```python
from build123d import *

# Parameters (mm, degrees)
SKETCH1_R           = 15
BOSS_EXTRUDE1_DEPTH = 300
SKETCH3_R           = 15
BOSS_EXTRUDE2_DEPTH = 50
BOSS_EXTRUDE3_START = -300
SKETCH5_R           = 15
BOSS_EXTRUDE3_DEPTH = 300


with BuildPart() as part:
    # Sketch1 → Boss-Extrude1 (new, symmetric)
    with BuildSketch(Plane.XY):
        Circle(SKETCH1_R)
    extrude(amount=BOSS_EXTRUDE1_DEPTH, both=True)

    # Sketch2 → Revolve1 (revolve)
    with BuildSketch(Plane(origin=(0, 0, 0), x_dir=(1, 0, 0), z_dir=(0, 1, 0))):
        with BuildLine():
            Line((0, 355), (0, 295))
            ThreePointArc((0, 295), (30, 325), (0, 355))
        make_face()
    revolve1 = revolve(axis=Axis((0, 0, -355), (0, 0, 1)))

    # Mirror1: Revolve1 across plane
    add(revolve1.mirror(Plane.XY))

    # Sketch3 → Boss-Extrude2 (add)
    with BuildSketch(Plane(origin=(0, 0, 0), x_dir=(1, 0, 0), z_dir=(0, 1, 0))):
        Circle(SKETCH3_R)
    extrude(amount=BOSS_EXTRUDE2_DEPTH)

    # Sketch4 → Revolve2 (revolve)
    with BuildSketch(Plane.XY):
        with BuildLine():
            Line((0, 105), (0, 45))
            ThreePointArc((0, 45), (30, 75), (0, 105))
        make_face()
    revolve(axis=Axis((0, 105, 0), (0, -1, 0)))

    # Sketch5 → Boss-Extrude3 (add)
    with BuildSketch(Plane(origin=(0, 0, 0), x_dir=(1, 0, 0), z_dir=(0, 1, 0)).offset(BOSS_EXTRUDE3_START)):
        Circle(SKETCH5_R)
    extrude(amount=BOSS_EXTRUDE3_DEPTH)

    # Sketch6 → Revolve3 (revolve)
    with BuildSketch(Plane(origin=(0, 0, 0), x_dir=(0, 0, -1), z_dir=(1, 0, 0))):
        with BuildLine():
            Line((0, -295), (0, -355))
            ThreePointArc((0, -355), (-30, -325), (0, -295))
        make_face()
    revolve(axis=Axis((0, -295, 0), (0, -1, 0)))


solid = part.part
```
Design review of the part built by this model. Coordinates are the model's own, in mm. Coordinates: 2 decimals unless noted, no trailing zeros. Order: outer loops, then holes, each group sorted by start corner. A loop starts at its lowest first (then second) coordinate and runs counter-clockwise, first axis right, second up.
1) Clearance check with flat-ended pins moving along their axes: pin 1 (12 mm diameter, centred on y = 2.5, z = -119, fed in from +X); pin 2 (6 mm diameter, centred on x = -6, z = -278.5, fed in from -Y); pin 3 (2 mm diameter, centred on x = 8, z = 62.5, fed in from +Y). State where each tip first meets the part, or that it passes through.
2) Take a section at B-B, the plane x = -22. Give the boundary of the cut face in (y, z), and give its area (3 significant figures).
3) Take a section at A-A, the plane y = -138. Give the boundary of the cut face in (x, z).
4) Wall thickness on line 1 along Y through (x, z) = (13, -13); line 2 along Y through (x, z) = (0, -163); line 3 along Z through (x, y) = (21.5, 1.5): over which ranges is each line inside the solid? List them lowest first.
Returned:
1. pin 1: stops at x = 15
1. pin 2: stops at y = -14.7
1. pin 3: stops at y = 13.27
2. outline: circle Ø40.79 at (-325, 0); circle Ø40.79 at (0, -325); circle Ø40.79 at (0, 325); circle Ø40.79 at (75, 0)
2. area: 5,230 mm2
3. outline: circle Ø30 at (0, 0)
4. line 1: y = -348.71 to -301.29, -7.48 to 7.48, 51.29 to 98.71
4. line 2: y = -15 to 15
4. line 3: z = -345.87 to -304.13, 304.13 to 345.87
